```python
from build123d import *

# Parameters (mm, degrees)
BOSS_EXTRUDE1_DEPTH = 200
SKETCH4_W           = 20
SKETCH4_H           = 250
BOSS_EXTRUDE2_DEPTH = 30
SKETCH5_R           = 5
CUT_EXTRUDE1_DEPTH  = 230
BOSS_EXTRUDE5_START = -60
BOSS_EXTRUDE5_DEPTH = 70


with BuildPart() as part:
    # Sketch2 → Boss-Extrude1 (new body)
    with BuildSketch(Plane.XY):
        Polygon((-148.050188004, -835.198427503), (-178.050188004, -835.198427503), (-178.050188004, -1405.198427503), (-1448.050188004, -1405.198427503), (-1448.050188004, -1435.198427503), (-148.050188004, -1435.198427503), align=None)
    extrude(amount=-BOSS_EXTRUDE1_DEPTH)

    # Sketch4 → Boss-Extrude2 (add)
    with BuildSketch(Plane.ZY.offset(1448.050188004)):
        with Locations((-190, -1420.198427503)):
            Rectangle(SKETCH4_W, SKETCH4_H)
        with Locations((-10, -1420.198427503)):
            Rectangle(SKETCH4_W, SKETCH4_H)
    extrude(amount=-BOSS_EXTRUDE2_DEPTH)

    # Sketch5 → Cut-Extrude1 (cut)
    with BuildSketch(Plane(origin=(0, 0, -200), x_dir=(-1, 0, 0), z_dir=(0, 0, -1))):
        with Locations((1433.050188004, -1320.198427503)):
            Circle(SKETCH5_R)
        with Locations((1433.050188004, -1373.198427503)):
            Circle(SKETCH5_R)
        with Locations((1433.050188004, -1520.198427503)):
            Circle(SKETCH5_R)
        with Locations((1433.050188004, -1467.198427503)):
            Circle(SKETCH5_R)
    extrude(amount=-CUT_EXTRUDE1_DEPTH, mode=Mode.SUBTRACT)

    # Sketch9 → Boss-Extrude5 (add)
    with BuildSketch(Plane.XY.offset(BOSS_EXTRUDE5_START)):
        with BuildLine():
            Line((-568.050188004, -1405.198427503), (-628.050188004, -1405.198427503))
            Line((-628.050188004, -1405.198427503), (-628.050188004, -635.198427503))
            ThreePointArc((-628.050188004, -635.198427503), (-598.050188004, -605.198427503), (-568.050188004, -635.198427503))
            Line((-568.050188004, -635.198427503), (-568.050188004, -1405.198427503))
        make_face()
    extrude(amount=-BOSS_EXTRUDE5_DEPTH)


solid = part.part
```
Part model, mm, in its own coordinate system. A direction names the side the tool comes from. Give positions to 0.01 mm unless a question says otherwise; leave off trailing zeros. Order: outer loops, then holes, each group sorted by start corner. A loop starts at its lowest first (then second) coordinate and runs counter-clockwise, first axis right, second up. Notation, with made-up numbers: M 41,42.5 L 66,42.5 A15 ccw 66,53.5 Z; hole C 71,57 d8. An arc over 180 degrees is marked long. Use a Markdown table: item, result. Add a question column.
(1) Saw through at D-D, the plane y = -812. Give the cut face in (x, z), and give its area (3 significant figures).
(2) Probe line 1 along X through (y, z) = (-923.5, -116.5); line 2 along X through (y, z) = (-1093, -151); line 3 along X through (y, z) = (-653.5, -117.5). List the from-to ranges inside material, lowest first. Write a range as [from, to].
(3) Saw through at A-A, the plane y = -1181. Give the cut face in (x, z).
(4) Mould opens along X. For faces 5 (the face through (-1433, -1491, -20)), 6 (the face through (-148.05, -1139, -99)), 7 (the face through (-568.05, -1015, -95)) say: +X half, -X half, draft (parallel to the pull), parting line (faces both ways), or undercut.
(5) 3-axis set-ups, long thin cutter, end or side, ignore diameter. For faces 1 (the face through (-1433, -1351, -20)), 2 (the face through (-1433, -1491, -180)), 3 (the face through (-163, -835.198, -99)), 4 (the face through (-598, -1000, -130)): which of +Z, -Z, +X, -X, +Y, -Y reach the whole face in a straight line?
(6) Drop flat-ended pins along their axis: P1, Ø1.5, axis at y = -1316, z = -89, coming from the -X side; P2, Ø8, axis at x = -692.5, z = -135, coming from the +Y side; P3, Ø6, axis at y = -1506.5, z = -190.5, coming from the +X side; P4, Ø9, axis at x = -1433.05, y = -1467.2, coming from the +Z side. Give the stop position or say it passes through.
(7) Saw through at B-B, the plane z = -73. Give the cut face in (x, y), and give its area (3 significant figures).
(8) Saw through at C-C, the plane x = -1046. Give the cut face in (y, z), and give its area (3 significant figures).
Answer key:
| question | item | result |
|---|---|---|
| 1 | outline | M -628.05,-130 L -568.05,-130 L -568.05,-60 L -628.05,-60 Z |
| 1 | area | 4,200 mm^2 |
| 2 | line 1 | [-628.05, -568.05], [-178.05, -148.05] |
| 2 | line 2 | [-178.05, -148.05] |
| 2 | line 3 | [-628.05, -568.05] |
| 3 | outline | M -628.05,-130 L -568.05,-130 L -568.05,-60 L -628.05,-60 Z; M -178.05,-200 L -148.05,-200 L -148.05,0 L -178.05,0 Z |
| 4 | face 5 | draft |
| 4 | face 6 | +X half |
| 4 | face 7 | undercut |
| 5 | face 1 | -X, +Y |
| 5 | face 2 | +X, -X, -Y |
| 5 | face 3 | +Z, -Z, +X, +Y |
| 5 | face 4 | -Z, -X, +Y |
| 6 | P1 | x = -628.05 |
| 6 | P2 | y = -1405.2 |
| 6 | P3 | x = -1418.05 |
| 6 | P4 | through |
| 7 | outline | M -1448.05,-1435.2 L -148.05,-1435.2 L -148.05,-835.2 L -178.05,-835.2 L -178.05,-1405.2 L -568.05,-1405.2 L -568.05,-635.2 A30 ccw -628.05,-635.2 L -628.05,-1405.2 L -1448.05,-1405.2 Z |
| 7 | area | 104,000 mm^2 |
| 8 | outline | M -1435.2,-200 L -1405.2,-200 L -1405.2,0 L -1435.2,0 Z |
| 8 | area | 6,000 mm^2 |
